from build123d import *

# Parameters (mm, degrees)
BOSS_EXTRUDE1_DEPTH     = 3.4
SKETCH2_OUTSIDE_W       = 23.196
SKETCH2_OUTSIDE_H       = 24.744
SKETCH2_OUTSIDE_R       = 5
CUT_EXTRUDE1_DEPTH      = 6.8
CUT_EXTRUDE1_DRAFT      = -30
MIRROR1_COPY_1_SKETCH_W = 23.196
MIRROR1_COPY_1_SKETCH_H = 24.744
MIRROR1_COPY_1_SKETCH_R = 5
MIRROR1_COPY_1_DEPTH    = 6.8
MIRROR1_COPY_1_DRAFT    = -30
SKETCH3_R               = 4
CUT_EXTRUDE3_DEPTH      = 6.8


with BuildPart() as part:
    # Sketch1 → Boss-Extrude1 (new, symmetric)
    with BuildSketch(Plane.XY):
        Polygon((0, 5.773502692), (-5, 2.886751346), (-5, -2.886751346), (0, -5.773502692), (5, -2.886751346), (5, 2.886751346), align=None)
    extrude(amount=BOSS_EXTRUDE1_DEPTH, both=True)


with BuildPart() as cut_extrude1_tool:
    # Sketch2 outside → Cut-Extrude1 (with draft: the straight prism first)
    with BuildSketch(Plane.XY.offset(3.4)):
        Rectangle(SKETCH2_OUTSIDE_W, SKETCH2_OUTSIDE_H)
        Circle(SKETCH2_OUTSIDE_R, mode=Mode.SUBTRACT)
    extrude(amount=-CUT_EXTRUDE1_DEPTH)
    # Cut-Extrude1: the draft: its side faces are tilted about the plane it starts from
    cut_extrude1_sides = [cut_extrude1_tool.faces().sort_by_distance(p)[0] for p in [
        (0, -12.372, 0),
        (11.598, 0, 0),
        (0, 12.372, 0),
        (-11.598, 0, 0),
        (-5, 0, 0),
    ]]
    draft(cut_extrude1_sides, Plane.XY.offset(3.4), CUT_EXTRUDE1_DRAFT)


with BuildPart() as part_1:
    add(part.part)

    # Cut-Extrude1: cut by cut_extrude1_tool
    add(cut_extrude1_tool.part, mode=Mode.SUBTRACT)


with BuildPart() as mirror1_copy_1_tool:
    # Mirror1 copy 1 sketch → Mirror1 copy 1 (with draft: the straight prism first)
    with BuildSketch(Plane(origin=(0, 0, -3.4), x_dir=(1, 0, 0), z_dir=(0, 0, -1))):
        Rectangle(MIRROR1_COPY_1_SKETCH_W, MIRROR1_COPY_1_SKETCH_H)
        Circle(MIRROR1_COPY_1_SKETCH_R, mode=Mode.SUBTRACT)
    extrude(amount=-MIRROR1_COPY_1_DEPTH)
    # Mirror1 copy 1: the draft: its side faces are tilted about the plane it starts from
    mirror1_copy_1_sides = [mirror1_copy_1_tool.faces().sort_by_distance(p)[0] for p in [
        (0, -12.372, 0),
        (11.598, 0, 0),
        (0, 12.372, 0),
        (-11.598, 0, 0),
        (-5, 0, 0),
    ]]
    draft(mirror1_copy_1_sides, Plane(origin=(0, 0, -3.4), x_dir=(1, 0, 0), z_dir=(0, 0, -1)), MIRROR1_COPY_1_DRAFT)


with BuildPart() as part_2:
    add(part_1.part)

    # Mirror1 copy 1: cut by mirror1_copy_1_tool
    add(mirror1_copy_1_tool.part, mode=Mode.SUBTRACT)

    # Sketch3 → Cut-Extrude3 (cut)
    with BuildSketch(Plane.XY.offset(3.4)):
        Circle(SKETCH3_R)
    extrude(amount=-CUT_EXTRUDE3_DEPTH, mode=Mode.SUBTRACT)


solid = part_2.part
Input: part model. Units: mm. Frame: model coordinates. Coordinates: 2 decimals unless noted, no trailing zeros. Loops run counter-clockwise (first coordinate to the right, second up) from the corner with the lowest first, then second, coordinate; pieces in that order, holes last.
(1) Section A-A on z = -0.75. Return the cut outline in (x, y), then the cut area to 3 significant figures.
(2) First-contact query: pin 1 Ø3 at (x, y) = (-0.5, -1.5) entering from +Z. Flat tip, straight axial feed; report the tip coordinate or a pass-through.
(3) Material intervals for probe 1 along Y at (x, z) = (-2.25, -1.75); probe 2 along Y at (x, z) = (-3, 2.25); probe 3 along X at (y, z) = (2.25, -3), sorted ascending.
(4) Pull-direction query (X, two-part tool) for faces 1 (the face through (4.483, -2.603, 3.081)), 2 (the face through (-0.867, -3.905, 0.048)), 3 (the face through (-4.483, 2.603, 3.081)); classes: released by +X, released by -X, zero draft, split by the parting line, or undercut.
Data:
1. outline: (-5, -2.89) - (0, -5.77) - (5, -2.89) - (5, 2.89) - (0, 5.77) - (-5, 2.89) - close; hole circle Ø8 at (0, 0)
1. area: 36.3 mm2
2. pin 1: passes through
3. probe 1: y = -4.47 to -3.31, 3.31 to 4.47
3. probe 2: y = -4.04 to -2.65, 2.65 to 4.04
3. probe 3: x = -4.72 to -3.31, 3.31 to 4.72
4. face 1: released by +X
4. face 2: undercut
4. face 3: released by -X
